Here's how the part is built. I have some questions about the finished solid (model axes, mm). A direction names the side the tool comes from. Give positions to 0.01 mm unless a question says otherwise; leave off trailing zeros. Loops run counter-clockwise (first coordinate to the right, second up) from the corner with the lowest first, then second, coordinate; pieces in that order, holes last. Notation, with made-up numbers: (35.25, -38.75) - (94.25, -38.75) arc R21 cw to (94.25, -27.75) - close; hole circle Ø7 at (-25, 80.25). An arc over 180 degrees is marked (long way). Return JSON: item names as keys, results as strings. Group by question number.
(1) I need wall thicknesses on probe 1 along X at (y, z) = (-7.25, 0.5); probe 2 along X at (y, z) = (6.75, 8); probe 3 along Y at (x, z) = (-100, 3). Which ranges of each line are inside material? Lowest first, please. Write a range as [from, to].
(2) If we section it at A-A (z = 7.5): Please give me the cut outline in (x, y), then the cut area to 3 significant figures.
(3) If we mould it in two halves opening along X, with no side actions, what happens to faces 1 (the flat face through (0, 0, 0)), 2 (the cylindrical face through (-147.972, -1.172, -8.923)), 3 (the flat face through (-66, -5.2, -0.2))? For each: released by +X, released by -X, zero draft, split by the parting line, or undercut.
(4) If we section it at C-C (x = -38): Please give me the cut outline in (y, z), then the cut area to 3 significant figures.
(5) If we section it at B-B (y = -7.25): Please give me the cut outline in (x, z), then the cut area to 3 significant figures.
(6) For P1, Ø1, axis at x = -65, y = -1.5, coming from the +Z side; P2, Ø3, axis at x = -37.5, y = -3.5, coming from the -Z side; P3, Ø5, axis at x = -15.5, z = 5, coming from the +Y side, each with a flat end and sliding along its axis, tell me the tip position at first contact or that it passes through.
(7) If we section it at D-D (z = 0): Please give me the cut outline in (x, y), then the cut area to 3 significant figures.
(8) On a 3-axis mill with a long thin cutter (end or side, diameter ignored), from which of +Z, -Z, +X, -X, +Y, -Y can I reach the whole of each face in a straight line? I mean faces 4 (the cylindrical face through (-105.44, -1.08, 4.88)), 5 (the flat face through (-150, 0, 0)), 6 (the cylindrical face through (-32.06, -1.08, 4.88)). Say none if no direction works.
```python
from build123d import *

# Parameters (mm, degrees)
EDGE_FILLET_R1_R = 1


with BuildPart() as part:
    # Shaft Profile Sketch → Shaft Body Revolve (revolve)
    with BuildSketch(Plane.XY):
        Polygon((-150, 0), (-150, 9), (-146, 9), (-146, 5), (-66, 5), (-66, 12), (-64, 12), (-64, 5), (0, 5), (0, 0), align=None)
    revolve(axis=Axis((0, 0, 0), (-1, 0, 0)))

    # Edge Fillet R1
    edge_fillet_r1_edges = [part.edges().sort_by_distance(p)[0] for p in [
        (0, -5, 0),
    ]]
    fillet(edge_fillet_r1_edges, radius=EDGE_FILLET_R1_R)


solid = part.part
```
Values:
{
 "1": {"probe 1": "[-150, -146], [-66, -64]", "probe 2": "[-66, -64]", "probe 3": "[-4, 4]"},
 "2": {"outline": "(-150, -4.97) - (-146, -4.97) - (-146, 4.97) - (-150, 4.97) - close; (-66, -9.37) - (-64, -9.37) - (-64, 9.37) - (-66, 9.37) - close", "area": "77.3 mm2"},
 "3": {"face 1": "released by +X", "face 2": "zero draft", "face 3": "undercut"},
 "4": {"outline": "circle Ø10 at (0, 0)", "area": "78.5 mm2"},
 "5": {"outline": "(-150, -5.33) - (-146, -5.33) - (-146, 5.33) - (-150, 5.33) - close; (-66, -9.56) - (-64, -9.56) - (-64, 9.56) - (-66, 9.56) - close", "area": "80.9 mm2"},
 "6": {"P1": "z = 11.96", "P2": "z = -4.58", "P3": "y = 4.33"},
 "7": {"outline": "(-150, -9) - (-146, -9) - (-146, -5) - (-66, -5) - (-66, -12) - (-64, -12) - (-64, -5) - (-1, -5) arc R1 ccw to (0, -4) - (0, 4) arc R1 ccw to (-1, 5) - (-64, 5) - (-64, 12) - (-66, 12) - (-66, 5) - (-146, 5) - (-146, 9) - (-150, 9) - close", "area": "1,560 mm2"},
 "8": {"face 4": "none", "face 5": "+Z, -Z, -X, +Y, -Y", "face 6": "+X"}
}
